Design review of the part built by this model. Coordinates are the model's own, in mm. A direction names the side the tool comes from. Give positions to 0.01 mm unless a question says otherwise; leave off trailing zeros. Write each loop counter-clockwise with the first axis right and the second up, starting at its lowest first coordinate (ties: lowest second). Pieces come first, ordered by that corner, then holes. Notation, with made-up numbers: M -37,46 L -24,46 A10 cw -24,65 Z; hole C 72.25,1 d5. An arc over 180 degrees is marked long. Use one line per item in the form item = value. Start each with the question number.
from build123d import *

# Parameters (mm, degrees)
SKETCH1_W           = 260
SKETCH1_H           = 20
BOSS_EXTRUDE1_DEPTH = 12.5
SKETCH2_R           = 3
CUT_EXTRUDE1_DEPTH  = 133.759180474
SKETCH3_W           = 20
SKETCH3_H           = 20
CUT_EXTRUDE2_DEPTH  = 8.5
CHAMFER1_SIZE       = 5
SKETCH4_R           = 3
BOSS_EXTRUDE2_DEPTH = 4
LPATTERN1_COUNT     = 2
LPATTERN1_PITCH     = 15


with BuildPart() as part:
    # Sketch1 → Boss-Extrude1 (new, symmetric)
    with BuildSketch(Plane.XY):
        Rectangle(SKETCH1_W, SKETCH1_H)
    extrude(amount=BOSS_EXTRUDE1_DEPTH, both=True)

    # Sketch2 → Cut-Extrude1 (cut, through all)
    with BuildSketch(Plane.XY.offset(12.5)):
        with Locations((-120, 0)):
            Circle(SKETCH2_R)
        with Locations((120, 0)):
            Circle(SKETCH2_R)
    extrude(amount=-CUT_EXTRUDE1_DEPTH, mode=Mode.SUBTRACT)

    # Sketch3 → Cut-Extrude2 (cut)
    with BuildSketch(Plane.XY.offset(12.5)):
        with Locations((-120, 0)):
            Rectangle(SKETCH3_W, SKETCH3_H)
        with Locations((120, 0)):
            Rectangle(SKETCH3_W, SKETCH3_H)
    cut_extrude2 = extrude(amount=-CUT_EXTRUDE2_DEPTH, mode=Mode.SUBTRACT)

    # Mirror2: Cut-Extrude2 across plane
    add(cut_extrude2.mirror(Plane.XY), mode=Mode.SUBTRACT)

    # Chamfer1
    chamfer1_edges = [part.edges().sort_by_distance(p)[0] for p in [
        (130, -10, 0),
        (-130, -10, 0),
        (-130, 10, 0),
        (130, 10, 0),
    ]]
    chamfer(chamfer1_edges, length=CHAMFER1_SIZE)

    # Sketch4 → Boss-Extrude2 (add)
    with BuildSketch(Plane(origin=(0, 0, -12.5), x_dir=(-1, 0, 0), z_dir=(0, 0, -1))):
        with BuildLine():
            Line((-46.5, -20), (-46.5, -10))
            Line((-46.5, -10), (-33.5, -10))
            Line((-33.5, -10), (-33.5, -20))
            ThreePointArc((-33.5, -20), (-40, -26.5), (-46.5, -20))
        make_face()
        with Locations((-40, -20)):
            Circle(SKETCH4_R, mode=Mode.SUBTRACT)
    boss_extrude2 = extrude(amount=-BOSS_EXTRUDE2_DEPTH)

    # LPattern1: Boss-Extrude2 ×2
    with Locations(*[(0, 0, i * LPATTERN1_PITCH) for i in range(1, LPATTERN1_COUNT)]):
        add(boss_extrude2)


solid = part.part
1. We need section C-C (x = -97). State the section outline as (y, z) points.
2. Clearance check with flat-ended pins moving along their axes: pin 1 Ø10.5 at (x, y) = (39, -18.5) entering from -Z; pin 2 Ø6 at (y, z) = (-20.5, 3) entering from +X; pin 3 Ø10.5 at (x, y) = (41.5, -16) entering from +Z; pin 4 Ø6 at (x, y) = (-121.5, 3.5) entering from -Z. State where each tip first meets the part, or that it passes through.
3. To check wall thickness, follow L1, parallel to Y at x = 40, z = -11.35; L2, parallel to Z at x = 38, y = -14; L3, parallel to Y at x = 120, z = -1. State the ranges of each line that lie inside material, in increasing order.
4. Draft analysis for pull direction X (two halves, no side actions). For faces 4 (the flat face through (128, -7, 0)), 5 (the cylindrical face through (-117.14, 0.9, 0.06)), 6 (the flat face through (-110, 0, 8)), 7 (the flat face through (-117.9, 2.4, -4)), state which applies: pulls with the +X half, pulls with the -X half, needs draft (parallel to the pull), parting line crosses it, or undercut.
5. We need section A-A (x = 120). State the section outline as (y, z) points, and give its area (3 significant figures).
6. We need section B-B (y = 0). State the section outline as (x, z) points, and give its area (3 significant figures).
7. For faces 1 (the flat face through (117.6, 2.4, -4)), 2 (the flat face through (40, -16, 6.5)), 3 (the flat face through (33.5, -15, -11)), list the 3-axis set-ups (+Z, -Z, +X, -X, +Y, -Y) from which the entire face can be reached by the end or side of a thin tool; tool diameter is ignored.
Answer block:
q1.outline = M -10,-12.5 L 10,-12.5 L 10,12.5 L -10,12.5 Z
q2.pin_1 = -12.5
q2.pin_2 = 46.5
q2.pin_3 = 6.5
q2.pin_4 = -4
q3.L1 = -26.5 to -23, -17 to 10
q3.L2 = -12.5 to -8.5, 2.5 to 6.5
q3.L3 = -10 to -3, 3 to 10
q4.face_4 = pulls with the +X half
q4.face_5 = undercut
q4.face_6 = pulls with the -X half
q4.face_7 = needs draft
q5.outline = M -10,-4 L -3,-4 L -3,4 L -10,4 Z; M 3,-4 L 10,-4 L 10,4 L 3,4 Z
q5.area = 112 mm^2
q6.outline = M -130,-4 L -123,-4 L -123,4 L -130,4 Z; M -117,-4 L -110,-4 L -110,-12.5 L 110,-12.5 L 110,-4 L 117,-4 L 117,4 L 110,4 L 110,12.5 L -110,12.5 L -110,4 L -117,4 Z; M 123,-4 L 130,-4 L 130,4 L 123,4 Z
q6.area = 5,720 mm^2
q7.face_1 = -Z, +X, +Y, -Y
q7.face_2 = +Z, +X, -X, -Y
q7.face_3 = +Z, -Z, -X, -Y
